Input: part model. Units: mm. Frame: model coordinates. Face numbers are marked on the shaded views. A direction names the side the tool comes from. Round coordinates to 2 decimals unless told otherwise and drop trailing zeros. Loops run counter-clockwise (first coordinate to the right, second up) from the corner with the lowest first, then second, coordinate; pieces in that order, holes last. Notation, with made-up numbers: M 37,-36 L 50,-36 A11 cw 50,-20 Z; hole C 88.25,88 d3. An arc over 180 degrees is marked long. Use one line per item in the form item = value. Start each with the question number.
Q1. Section query B-B, the plane x = -206. Output: boundary loops of the cut face in (y, z), and give its area (3 significant figures).
Q2. Mould query, pull axis X, two halves, no side actions, for the marked faces 1 and 2. Classes: pulls with the +X half, pulls with the -X half, needs draft (parallel to the pull), parting line crosses it, or undercut.
Q3. Section query D-D, the plane y = 167. Output: boundary loops of the cut face in (x, z), and give its area (3 significant figures).
Q4. Ray query, line 1 along Y through (x, z) = (-147.5, 2); line 2 along Y through (x, z) = (-185, 1.5); line 3 along Y through (x, z) = (-137, 4). Return the intervals inside material, ascending.
Q5. Access query for the marked faces 3 and 4. Directions: +Z, -Z, +X, -X, +Y, -Y. A direction counts if a zero-diameter tool reaches every point of the face in a straight line with its end or side. Return the directions, or none.
Q6. First-contact query: P1, Ø1.8, axis at x = -185.61, y = 197.47, coming from the -Z side; P2, Ø1.5, axis at y = 180, z = 6.5, coming from the +X side; P3, Ø2, axis at y = 187, z = 4, coming from the +X side; P4, Ø1, axis at x = -158.5, z = 4.5, coming from the +Y side. Flat tips, straight axial feed; report the tip coordinate or a pass-through.
Q7. Section query C-C, the plane x = -186. Output: boundary loops of the cut face in (y, z), and give its area (3 significant figures).
Q8. Section query A-A, the plane z = 6.75. State how many separate pieces and enclosed holes the cut face has, and give its area (3 significant figures).
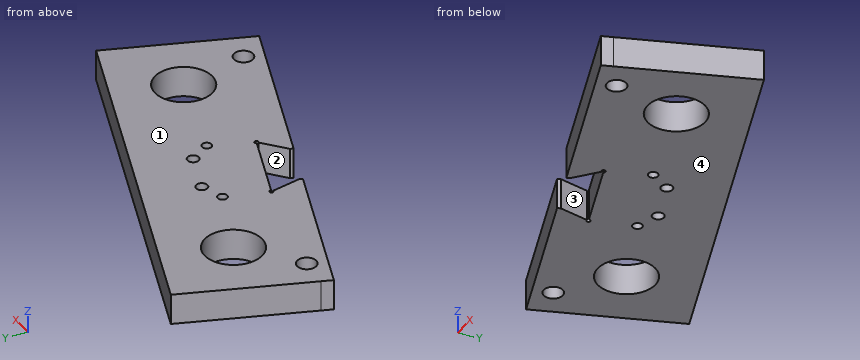
```python
from build123d import *

# Parameters (mm, degrees)
SKETCH_1_R             = 7.5
EXTRUDE_1_DEPTH        = 8
SKETCH_2_W             = 105
SKETCH_2_H             = 8
EXTRUDE_2_DEPTH        = 3
CUT_EXTRUDE_1_DEPTH    = 326.744737494
HOLE_WIZARD_M6_1_D     = 5
HOLE_WIZARD_M6_1_DEPTH = 15
HOLE_WIZARD_M6_1_TIP   = 1.502151548
HOLE_WIZARD_M3_1_D     = 2.5
MM_1_D                 = 3
CUT_EXTRUDE_2_DEPTH    = 10
SKETCH_14_R            = 0.5
CUT_EXTRUDE_3_DEPTH    = 326.744737494


with BuildPart() as part:
    # 草图1 → 凸台-拉伸1 (new body)
    with BuildSketch(Plane.XY):
        Polygon((-123.272913695, 191.443187885), (-134.630416513, 158.337189489), (-233.948411698, 192.409697944), (-222.59090888, 225.515696339), align=None)
        with Locations(Location((-211.716661092, 203.283945733, 0), (0, 0, 90))):
            Circle(SKETCH_1_R, mode=Mode.SUBTRACT)
        with Locations(Location((-145.504664302, 180.568940096, 0), (0, 0, 90))):
            Circle(SKETCH_1_R, mode=Mode.SUBTRACT)
    extrude(amount=EXTRUDE_1_DEPTH)

    # 草图2 → 凸台-拉伸2 (add)
    with BuildSketch(Plane(origin=(34.423389522, 100.340778821, 0), x_dir=(0.9458856684293921, -0.3245000805236912, 0), z_dir=(-0.3245000805236912, -0.9458856684293921, 0))):
        with Locations((-231.225412254, 4)):
            Rectangle(SKETCH_2_W, SKETCH_2_H)
    extrude(amount=EXTRUDE_2_DEPTH)

    # 草图3 → 切除-拉伸1 (cut, through all)
    with BuildSketch(Plane.XY.offset(8)):
        Polygon((-181.873786677, 171.373096295), (-193.224414699, 175.267097261), (-194.997272817, 184.33298428), (-174.908927271, 177.441379972), align=None)
    extrude(amount=-CUT_EXTRUDE_1_DEPTH, mode=Mode.SUBTRACT)

    # M6 螺纹孔1
    with Locations(Plane.XY.offset(8)):
        with Locations((-141.5485017, 162.824961471), (-225.73232619, 191.705468637)):
            Hole(HOLE_WIZARD_M6_1_D / 2, depth=HOLE_WIZARD_M6_1_DEPTH)
            with Locations((0, 0, -(HOLE_WIZARD_M6_1_DEPTH + HOLE_WIZARD_M6_1_TIP / 2))):  # 118° drill point
                Cone(0, HOLE_WIZARD_M6_1_D / 2, HOLE_WIZARD_M6_1_TIP, mode=Mode.SUBTRACT)

    # M3 螺纹孔1 (through all)
    with Locations(Plane(origin=(0, 0, 0), x_dir=(-1, 0, 0), z_dir=(0, 0, -1))):
        with Locations((170.819179959, 188.188267601), (191.635646748, 195.306884773)):
            Hole(HOLE_WIZARD_M3_1_D / 2)

    # 大小mm 暗销孔1 (through all)
    with Locations(Plane(origin=(0, 0, 0), x_dir=(-1, 0, 0), z_dir=(0, 0, -1))):
        with Locations((174.256171582, 193.590156353), (185.610608012, 197.473038447)):
            Hole(MM_1_D / 2)

    # 草图13 → 切除-拉伸2 (cut)
    with BuildSketch(Plane.XY.offset(8)):
        Polygon((-193.697357533, 175.429347302), (-192.732083432, 178.243025921), (-180.825057933, 172.889205286), (-181.400843843, 171.210846255), align=None)
    extrude(amount=-CUT_EXTRUDE_2_DEPTH, mode=Mode.SUBTRACT)

    # 草图14 → 切除-拉伸3 (cut, through all)
    with BuildSketch(Plane.XY.offset(8)):
        with Locations((-194.997272817, 184.33298428)):
            Circle(SKETCH_14_R)
        with Locations((-174.908927271, 177.441379972)):
            Circle(SKETCH_14_R)
    extrude(amount=-CUT_EXTRUDE_3_DEPTH, mode=Mode.SUBTRACT)


solid = part.part
```
Results found:
q1.outline = M 179.65,0 L 198.43,0 L 198.43,8 L 179.65,8 Z; M 208.14,0 L 219.82,0 L 219.82,8 L 208.14,8 Z
q1.area = 244 mm²
q2.face_1 = needs draft
q2.face_2 = undercut
q3.outline = M -169.13,0 L -131.66,0 L -131.66,8 L -169.13,8 Z
q3.area = 300 mm²
q4.line_1 = 159.58 to 173.34, 187.8 to 199.75
q4.line_2 = 180.9 to 196.1, 198.84 to 212.62
q4.line_3 = 155.98 to 196.15
q5.face_3 = +Z, -Z
q5.face_4 = -Z, +X, -X, +Y, -Y
q6.P1 = through
q6.P2 = -126.94
q6.P3 = -124.45
q6.P4 = 203.7
q7.outline = M 181.25,0 L 196.02,0 L 196.02,8 L 181.25,8 Z; M 198.92,0 L 212.96,0 L 212.96,8 L 198.92,8 Z
q7.area = 231 mm²
q8.separate_pieces = 1
q8.enclosed_holes = 8
q8.area = 3,440 mm²
